Design review of the part built by this model. Coordinates are the model's own, in mm. Face numbers are marked on the shaded views. A direction names the side the tool comes from. Give positions to 0.01 mm unless a question says otherwise; leave off trailing zeros. Loops run counter-clockwise (first coordinate to the right, second up) from the corner with the lowest first, then second, coordinate; pieces in that order, holes last. Notation, with made-up numbers: (7, -27) -> (43, -27) arc R28 cw to (43, -9) -> close; hole circle Ø2 at (-0.5, -19). An arc over 180 degrees is marked (long way). Use a Markdown table: item, result. Add a question column.
1. Add section C-C (y = -20). State the section outline as (x, z) points.
2. For pin 1 Ø1.5 at (y, z) = (-18, 3) entering from +X; pin 2 Ø2 at (x, z) = (-0.5, 2) entering from -Y; pin 3 Ø1.5 at (x, z) = (-10.5, 2.5) entering from -Y; pin 4 Ø2 at (x, z) = (-3.5, 2.5) entering from -Y, all flat-tipped, find the tip position at first contact; note any pin that passes through.
3. For the marked faces 1 and 2, list the 3-axis set-ups (+Z, -Z, +X, -X, +Y, -Y) from which the entire face can be reached by the end or side of a thin tool; tool diameter is ignored.
4. Draft analysis for pull direction X (two halves, no side actions). For the marked faces 3, 4, 5 and 6, state which applies: pulls with the +X half, pulls with the -X half, needs draft (parallel to the pull), parting line crosses it, or undercut.
5. Add section B-B (z = 1.9). State the section outline as (x, y) points, and give its area (3 significant figures).
6. Add section A-A (y = -3.5). State the section outline as (x, z) points.
7. To check wall thickness, follow line 1 (X direction, y = -11.5, z = 3.65); line 2 (X direction, y = -8, z = 0.65); line 3 (Y direction, x = 8, z = 1.2). State the ranges of each line that lie inside material, in increasing order.
```python
from build123d import *

# Parameters (mm, degrees)
CAM_PLATE_4MM_DEPTH       = 4
SLOTS_CUT_DEPTH           = 4
CSK_HOLE_M2_5_D           = 2.9
CSK_HOLE_M2_5_DEPTH       = 29
CSK_HOLE_M2_5_CSINK_D     = 5.5
CSK_HOLE_M2_5_CSINK_ANGLE = 90
CSK_HOLE_M2_5_TIP         = 0.871247898
CSK_HOLE_M2_D             = 2.4
CSK_HOLE_M2_DEPTH         = 29
CSK_HOLE_M2_CSINK_D       = 4.4
CSK_HOLE_M2_CSINK_ANGLE   = 90
CSK_HOLE_M2_TIP           = 0.721032743


with BuildPart() as part:
    # Cam Plate Profile Sketch → Cam Plate 4mm (new body)
    with BuildSketch(Plane.XY):
        with BuildLine():
            Line((4, 4.474241718), (-4, 4.474241718))
            Line((-4, 4.474241718), (-9, 2.474241718))
            Line((-9, 2.474241718), (-13.616491046, -10.209463189))
            ThreePointArc((-13.616491046, -10.209463189), (-13.146761684, -13.741504469), (-9.979750738, -15.374294397))
            ThreePointArc((-9.979750738, -15.374294397), (-7.940438794, -16.159442387), (-6.974754793, -18.11972425))
            ThreePointArc((-6.974754793, -18.11972425), (-4.735094414, -22.681229249), (0, -24.525758282))
            Line((0, -24.525758282), (6, -24.525758282))
            ThreePointArc((6, -24.525758282), (11.754495804, -22.083255744), (13.995148957, -16.247202791))
            Line((13.995148957, -16.247202791), (14, -13.525758282))
            Line((14, -13.525758282), (14, -9.356766198))
            ThreePointArc((14, -9.356766198), (13.881480036, -8.274568128), (13.531538935, -7.243674889))
            Line((13.531538935, -7.243674889), (9, 2.474241718))
            Line((9, 2.474241718), (4, 4.474241718))
        make_face()
    extrude(amount=CAM_PLATE_4MM_DEPTH)

    # Slot Profiles Sketch → Slots Cut (cut)
    with BuildSketch(Plane.XY.offset(4)):
        with BuildLine():
            Line((-2.5, -0.525758282), (2.5, -0.525758282))
            ThreePointArc((2.5, -0.525758282), (4.5, -2.525758282), (2.5, -4.525758282))
            Line((2.5, -4.525758282), (-2.5, -4.525758282))
            ThreePointArc((-2.5, -4.525758282), (-4.5, -2.525758282), (-2.5, -0.525758282))
        make_face()
        with BuildLine():
            Line((5.101968483, -7.445469013), (6.395655964, -5.90371231))
            ThreePointArc((6.395655964, -5.90371231), (7.124526222, -5.547191119), (7.877870447, -5.848574084))
            ThreePointArc((7.877870447, -5.848574084), (9.969385657, -8.876957403), (10.944861808, -12.425758282))
            ThreePointArc((10.944861808, -12.425758282), (10.69149422, -13.196578675), (9.949874371, -13.525758282))
            Line((9.949874371, -13.525758282), (7.937253933, -13.525758282))
            ThreePointArc((7.937253933, -13.525758282), (7.275816105, -13.275758282), (6.945097192, -12.650758282))
            ThreePointArc((6.945097192, -12.650758282), (6.344154509, -10.56743045), (5.134511311, -8.76794433))
            ThreePointArc((5.134511311, -8.76794433), (4.868315554, -8.112856688), (5.101968483, -7.445469013))
        make_face()
    extrude(amount=-SLOTS_CUT_DEPTH, mode=Mode.SUBTRACT)

    # CSK Hole M2.5
    with Locations(Plane(origin=(0, -13.525758282, 4), x_dir=(1, 0, 0), z_dir=(0, 0, 1))):
        with Locations((0, 0)):
            CounterSinkHole(CSK_HOLE_M2_5_D / 2, CSK_HOLE_M2_5_CSINK_D / 2, depth=CSK_HOLE_M2_5_DEPTH, counter_sink_angle=CSK_HOLE_M2_5_CSINK_ANGLE)
            with Locations((0, 0, -(CSK_HOLE_M2_5_DEPTH + CSK_HOLE_M2_5_TIP / 2))):  # 118° drill point
                Cone(0, CSK_HOLE_M2_5_D / 2, CSK_HOLE_M2_5_TIP, mode=Mode.SUBTRACT)

    # CSK Hole M2
    with Locations(Plane(origin=(-7, -7.525758282, 4), x_dir=(1, 0, 0), z_dir=(0, 0, 1))):
        with Locations((0, 0)):
            CounterSinkHole(CSK_HOLE_M2_D / 2, CSK_HOLE_M2_CSINK_D / 2, depth=CSK_HOLE_M2_DEPTH, counter_sink_angle=CSK_HOLE_M2_CSINK_ANGLE)
            with Locations((0, 0, -(CSK_HOLE_M2_DEPTH + CSK_HOLE_M2_TIP / 2))):  # 118° drill point
                Cone(0, CSK_HOLE_M2_D / 2, CSK_HOLE_M2_TIP, mode=Mode.SUBTRACT)


solid = part.part
```
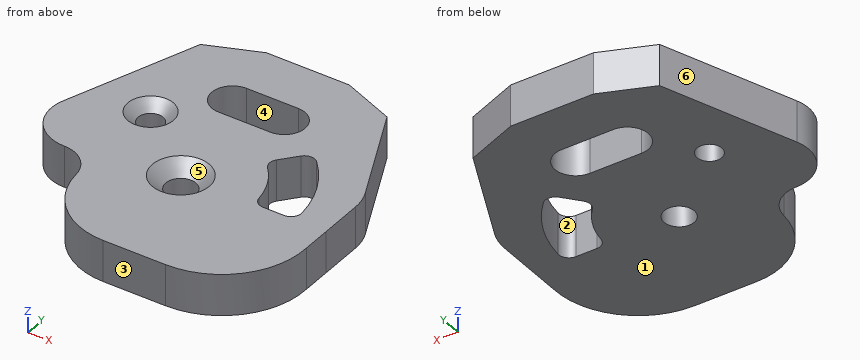
Taken from the geometry:
| question | item | result |
|---|---|---|
| 1 | outline | (-6.55, 0) -> (13.21, 0) -> (13.21, 4) -> (-6.55, 4) -> close |
| 2 | pin 1 | stops at x = 13.97 |
| 2 | pin 2 | stops at y = -24.53 |
| 2 | pin 3 | stops at y = -15.38 |
| 2 | pin 4 | stops at y = -24.06 |
| 3 | face 1 | -Z, +X, -X, +Y, -Y |
| 3 | face 2 | +Z, -Z |
| 4 | face 3 | needs draft |
| 4 | face 4 | undercut |
| 4 | face 5 | undercut |
| 4 | face 6 | pulls with the -X half |
| 5 | outline | (-13.62, -10.21) arc R3.85 ccw to (-9.98, -15.37) arc R3 cw to (-6.97, -18.12) arc R7 ccw to (0, -24.53) -> (6, -24.53) arc R8 ccw to (14, -16.25) -> (14, -13.53) -> (14, -9.36) arc R5 ccw to (13.53, -7.24) -> (9, 2.47) -> (4, 4.47) -> (-4, 4.47) -> (-9, 2.47) -> close; hole circle Ø2.4 at (-7, -7.53); hole (-2.5, -4.53) -> (2.5, -4.53) arc R2 ccw to (2.5, -0.53) -> (-2.5, -0.53) arc R2 ccw to start; hole circle Ø2.9 at (0, -13.53); hole (5.1, -7.45) arc R1 ccw to (5.13, -8.77) arc R7 cw to (6.95, -12.65) arc R1 ccw to (7.94, -13.53) -> (9.95, -13.53) arc R1 ccw to (10.94, -12.43) arc R11 ccw to (7.88, -5.85) arc R1 ccw to (6.4, -5.9) -> close |
| 5 | area | 556 mm^2 |
| 6 | outline | (-11.17, 0) -> (-4.25, 0) -> (-4.25, 4) -> (-11.17, 4) -> close; (4.25, 0) -> (11.79, 0) -> (11.79, 4) -> (4.25, 4) -> close |
| 7 | line 1 | x = -13.85 to -1.29, 1.29 to 6.7, 10.81 to 14 |
| 7 | line 2 | x = -12.81 to -8.1, -5.9 to 4.87, 9.51 to 13.81 |
| 7 | line 3 | y = -24.27 to -13.53, -5.98 to 2.87 |
